Model file for the job. Use its own axes, mm. Round coordinates to 2 decimals unless told otherwise and drop trailing zeros. Write each loop counter-clockwise with the first axis right and the second up, starting at its lowest first coordinate (ties: lowest second). Pieces come first, ordered by that corner, then holes. Notation, with made-up numbers: (21.5, -8.5) - (32.5, -8.5) arc R6 cw to (32.5, 1.5) - close; hole circle Ø3 at (87.25, 56.25). An arc over 180 degrees is marked (long way). Answer as a JSON object with one key per item and string values. Group by question number.
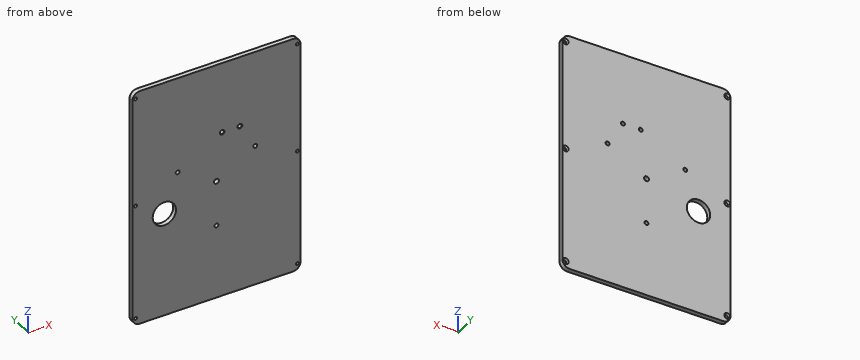
from build123d import *

# Parameters (mm, degrees)
SKETCH1_W                                       = 180
SKETCH1_H                                       = 252
BOSS_EXTRUDE1_DEPTH                             = 5
SKETCH2_R                                       = 70
BOSS_EXTRUDE2_DEPTH                             = 50
DOME1_FACE_RADIUS                               = 70
DOME1_HEIGHT                                    = 50
SKETCH3_R                                       = 2.1
CUT_EXTRUDE1_DEPTH                              = 188.085541932
CSK_FOR_M3_FLAT_HEAD_MACHINE_SCREW1_D           = 3.2
CSK_FOR_M3_FLAT_HEAD_MACHINE_SCREW1_DEPTH       = 8.5
CSK_FOR_M3_FLAT_HEAD_MACHINE_SCREW1_CSINK_D     = 6.3
CSK_FOR_M3_FLAT_HEAD_MACHINE_SCREW1_CSINK_ANGLE = 90
CSK_FOR_M3_FLAT_HEAD_MACHINE_SCREW1_TIP         = 0.96137699
SKETCH7_R                                       = 2.6
CUT_EXTRUDE3_DEPTH                              = 15
SKETCH9_W                                       = 180
SKETCH9_H                                       = 252
CUT_EXTRUDE4_DEPTH                              = 168
SKETCH11_R                                      = 12.5
CUT_EXTRUDE5_DEPTH                              = 49
FILLET1_R                                       = 8
M5_TAPPED_HOLE1_D                               = 4.2
M5_TAPPED_HOLE1_DEPTH                           = 14
M5_TAPPED_HOLE1_CSINK_D                         = 5.05
M5_TAPPED_HOLE1_CSINK_ANGLE                     = 90
M5_TAPPED_HOLE1_TIP                             = 1.2618073


with BuildPart() as part:
    # Sketch1 → Boss-Extrude1 (new body)
    with BuildSketch(Plane(origin=(0, 0, 0), x_dir=(1, 0, 0), z_dir=(0, 1, 0))):
        Rectangle(SKETCH1_W, SKETCH1_H)
    extrude(amount=BOSS_EXTRUDE1_DEPTH)

    # Sketch2 → Boss-Extrude2 (add)
    with BuildSketch(Plane(origin=(0, 5, 0), x_dir=(1, 0, 0), z_dir=(0, 1, 0))):
        with Locations(Location((0, 0, 0), (0, 0, 270))):
            Circle(SKETCH2_R)
    extrude(amount=BOSS_EXTRUDE2_DEPTH)

    # Dome1: a dome of height H over a round flat face of radius A is a cap of a sphere of radius (A * A + H * H) / (2 * H)
    dome1_r = (DOME1_FACE_RADIUS * DOME1_FACE_RADIUS + DOME1_HEIGHT * DOME1_HEIGHT) / (2 * DOME1_HEIGHT)
    dome1_base = Plane((0, 55, 0), z_dir=(0, 1, 0))
    with Locations(dome1_base.offset(DOME1_HEIGHT - dome1_r)):
        dome1_ball = Sphere(dome1_r, mode=Mode.PRIVATE)
    add(split(dome1_ball, bisect_by=dome1_base, keep=Keep.TOP, mode=Mode.PRIVATE))

    # Sketch3 → Cut-Extrude1 (cut, through all)
    with BuildSketch(Plane.XZ):
        with Locations(Location((0, -48, 0), (0, 0, 270))):
            Circle(SKETCH3_R)
        with Locations(Location((-41.569219382, 24, 0), (0, 0, 270))):
            Circle(SKETCH3_R)
        with Locations(Location((41.569219382, 24, 0), (0, 0, 270))):
            Circle(SKETCH3_R)
    extrude(amount=-CUT_EXTRUDE1_DEPTH, mode=Mode.SUBTRACT)

    # CSK for M3 Flat Head Machine Screw1
    with Locations(Plane(origin=(0, 5, 0), x_dir=(1, 0, 0), z_dir=(0, 1, 0))):
        with Locations((86.5, 119), (86.5, -3), (86.5, -119), (-86.5, -119), (-86.5, -3), (-86.5, 119)):
            CounterSinkHole(CSK_FOR_M3_FLAT_HEAD_MACHINE_SCREW1_D / 2, CSK_FOR_M3_FLAT_HEAD_MACHINE_SCREW1_CSINK_D / 2, depth=CSK_FOR_M3_FLAT_HEAD_MACHINE_SCREW1_DEPTH, counter_sink_angle=CSK_FOR_M3_FLAT_HEAD_MACHINE_SCREW1_CSINK_ANGLE)
            with Locations((0, 0, -(CSK_FOR_M3_FLAT_HEAD_MACHINE_SCREW1_DEPTH + CSK_FOR_M3_FLAT_HEAD_MACHINE_SCREW1_TIP / 2))):  # 118° drill point
                Cone(0, CSK_FOR_M3_FLAT_HEAD_MACHINE_SCREW1_D / 2, CSK_FOR_M3_FLAT_HEAD_MACHINE_SCREW1_TIP, mode=Mode.SUBTRACT)

    # Sketch7 → Cut-Extrude3 (cut)
    with BuildSketch(Plane.XZ):
        with Locations(Location((0, 0, 0), (0, 0, 270))):
            Circle(SKETCH7_R)
    extrude(amount=-CUT_EXTRUDE3_DEPTH, mode=Mode.SUBTRACT)

    # Sketch9 → Cut-Extrude4 (cut)
    with BuildSketch(Plane(origin=(0, 5, 0), x_dir=(1, 0, 0), z_dir=(0, 1, 0))):
        Rectangle(SKETCH9_W, SKETCH9_H)
    extrude(amount=CUT_EXTRUDE4_DEPTH, mode=Mode.SUBTRACT)

    # Sketch11 → Cut-Extrude5 (cut)
    with BuildSketch(Plane(origin=(0, 5, 0), x_dir=(1, 0, 0), z_dir=(0, 1, 0))):
        with Locations(Location((-55.749439459, 16, 0), (0, 0, 270))):
            Circle(SKETCH11_R)
    extrude(amount=-CUT_EXTRUDE5_DEPTH, mode=Mode.SUBTRACT)

    # Fillet1
    fillet1_edges = [part.edges().sort_by_distance(p)[0] for p in [
        (90, 2.5, 126),
        (-90, 2.5, 126),
        (-90, 2.5, -126),
        (90, 2.5, -126),
    ]]
    fillet(fillet1_edges, radius=FILLET1_R)

    # M5 Tapped Hole1
    with Locations(Plane(origin=(0, 0, 0), x_dir=(-1, 0, 0), z_dir=(0, -1, 0))):
        with Locations((-25.121103622, -51), (-6.121103622, -51)):
            CounterSinkHole(M5_TAPPED_HOLE1_D / 2, M5_TAPPED_HOLE1_CSINK_D / 2, depth=M5_TAPPED_HOLE1_DEPTH, counter_sink_angle=M5_TAPPED_HOLE1_CSINK_ANGLE)
            with Locations((0, 0, -(M5_TAPPED_HOLE1_DEPTH + M5_TAPPED_HOLE1_TIP / 2))):  # 118° drill point
                Cone(0, M5_TAPPED_HOLE1_D / 2, M5_TAPPED_HOLE1_TIP, mode=Mode.SUBTRACT)


solid = part.part
(1) Slice it at A-A (z = -16). Write the cut outline in (x, y), then the cut area to 3 significant figures.
(2) Flat gauge pins, fed straight in: pin 1 (6.5 mm diameter, centred on x = 25.12, z = 51, fed in from +Y); pin 2 (1.9 mm diameter, centred on x = 86.5, z = 3, fed in from -Y); pin 3 (4 mm diameter, centred on x = 86.5, z = -119, fed in from +Y). Where does each tip first touch, or does it go through?
(3) Drill centre lines: line 1 (X direction, y = 3.8, z = 51); line 2 (X direction, y = 3.25, z = -48); line 3 (Z direction, x = -86.5, y = 1.35). Where is each one in solid material? Low to high. Write a range as from..to.
(4) Slice it at B-B (y = 1.9). Count the separate pieces of the cut face and the enclosed holes in it, then the cut area to 3 significant figures.
Answer:
{
 "1": {"outline": "(-90, 0) - (-68.25, 0) - (-68.25, 5) - (-90, 5) - close; (-43.25, 0) - (90, 0) - (90, 5) - (-43.25, 5) - close", "area": "775 mm²"},
 "2": {"pin 1": "y = 5", "pin 2": "through", "pin 3": "y = 3.85"},
 "3": {"line 1": "-90..4.02, 8.22..23.02, 27.22..90", "line 2": "-90..-2.1, 2.1..90", "line 3": "-124.61..-120.6, -117.4..1.4, 4.6..117.4, 120.6..124.61"},
 "4": {"separate pieces": "1", "enclosed holes": "13", "area": "44,700 mm²"}
}
